Here's how the part is built. I have some questions about the finished solid (model axes, mm). Face numbers are marked on the shaded views. Give positions to 0.01 mm unless a question says otherwise; leave off trailing zeros. Write each loop counter-clockwise with the first axis right and the second up, starting at its lowest first coordinate (ties: lowest second). Pieces come first, ordered by that corner, then holes. Notation, with made-up numbers: (52, 54) - (90, 54) arc R25 ccw to (90, 72) - close; hole circle Ø4 at (-1, 62). An arc over 180 degrees is marked (long way). Use one line per item in the form item = value. Start each with the question number.
from build123d import *

# Parameters (mm, degrees)
BOSS_EXTRUDE1_DEPTH = 457.2
CUT_EXTRUDE1_REACH  = 460.697
SKETCH2_W           = 33.274
SKETCH2_H           = 15.85
CUT_EXTRUDE2_DEPTH  = 459.696855232


with BuildPart() as part:
    # Sketch1 → Boss-Extrude1 (new body)
    with BuildSketch(Plane.XY):
        with BuildLine():
            Line((30.25, 3.1), (30.25, 19.05))
            Line((30.25, 19.05), (31.75, 19.05))
            Line((31.75, 19.05), (31.75, 3.2))
            ThreePointArc((31.75, 3.2), (30.8127417, 0.9372583), (28.55, 0))
            Line((28.55, 0), (3.2, 0))
            ThreePointArc((3.2, 0), (0.9372583, 0.9372583), (0, 3.2))
            Line((0, 3.2), (0, 19.05))
            Line((0, 19.05), (1.5, 19.05))
            Line((1.5, 19.05), (1.5, 3.1))
            ThreePointArc((1.5, 3.1), (1.96862915, 1.96862915), (3.1, 1.5))
            Line((3.1, 1.5), (28.65, 1.5))
            ThreePointArc((28.65, 1.5), (29.78137085, 1.96862915), (30.25, 3.1))
        make_face()
    extrude(amount=BOSS_EXTRUDE1_DEPTH)

    # Sketch2 → Cut-Extrude1 (cut, up to next)
    with BuildSketch(Plane.ZY, mode=Mode.PRIVATE) as cut_extrude1_sk1:
        with Locations((156.337, 11.125)):
            Rectangle(SKETCH2_W, SKETCH2_H)
    cut_extrude1_tool1 = extrude(cut_extrude1_sk1.sketch, amount=-CUT_EXTRUDE1_REACH, mode=Mode.PRIVATE) & part.part
    add(cut_extrude1_tool1.solids().sort_by_distance((0, 11.125, 156.337))[0], mode=Mode.SUBTRACT)

    # Sketch4 → Cut-Extrude2 (cut, through all)
    with BuildSketch(Plane.XZ):
        with BuildLine():
            Line((9.525, 457.2), (9.525, 438.15))
            ThreePointArc((9.525, 438.15), (15.875, 431.8), (22.225, 438.15))
            Line((22.225, 438.15), (22.225, 457.2))
            Line((22.225, 457.2), (9.525, 457.2))
        make_face()
    cut_extrude2 = extrude(amount=-CUT_EXTRUDE2_DEPTH, mode=Mode.SUBTRACT)

    # Mirror1: Cut-Extrude2 across plane
    add(cut_extrude2.mirror(Plane.XY.offset(228.6)), mode=Mode.SUBTRACT)


solid = part.part
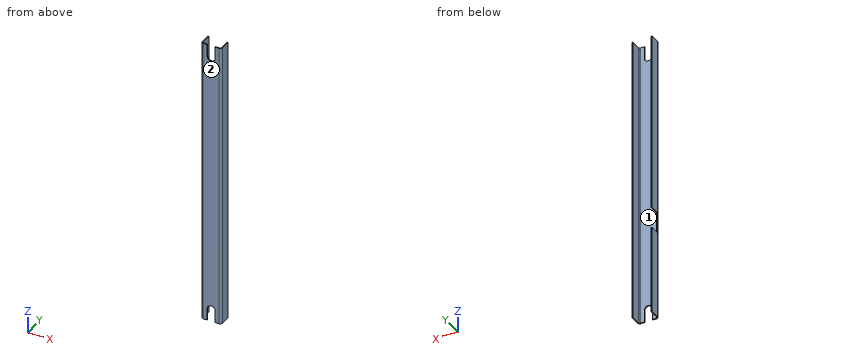
1. I want a section at B-B, the plane z = 198. List the corners of the cut face in (x, y) for me.
2. I want a section at A-A, the plane y = 15.75. List the corners of the cut face in (x, z) for me.
3. Please list where these lines run through material, in increasing order: line 1 (X direction, y = 9.75, z = 383); line 2 (Y direction, x = 20.5, z = 386); line 3 (X direction, y = 12.25, z = 161).
4. For P1, Ø0.8, axis at x = 1, z = 153.5, coming from the +Y side; P2, Ø8, axis at y = 10.5, z = 156, coming from the -X side; P3, Ø1.2, axis at y = 0.5, z = 447.5, coming from the -X side, each with a flat end and sliding along its axis, tell me the tip position at first contact or that it passes through.
5. We'd pull the mould along X, two halves only. Please class the marked faces 1 and 2: pulls with the +X half, pulls with the -X half, needs draft (parallel to the pull), parting line crosses it, or undercut.
Result sheet:
q1.outline = (0, 3.2) arc R3.2 ccw to (3.2, 0) - (28.55, 0) arc R3.2 ccw to (31.75, 3.2) - (31.75, 19.05) - (30.25, 19.05) - (30.25, 3.1) arc R1.6 cw to (28.65, 1.5) - (3.1, 1.5) arc R1.6 cw to (1.5, 3.1) - (1.5, 19.05) - (0, 19.05) - close
q2.outline = (0, 0) - (1.5, 0) - (1.5, 139.7) - (0, 139.7) - close; (0, 172.97) - (1.5, 172.97) - (1.5, 457.2) - (0, 457.2) - close; (30.25, 0) - (31.75, 0) - (31.75, 457.2) - (30.25, 457.2) - close
q3.line_1 = 0 to 1.5, 30.25 to 31.75
q3.line_2 = 0 to 1.5
q3.line_3 = 30.25 to 31.75
q4.P1 = 3.2
q4.P2 = 30.25
q4.P3 = 0.79
q5.face_1 = undercut
q5.face_2 = needs draft
